Verification items for the finished model (mm, model axes). Give positions to 0.01 mm unless a question says otherwise; leave off trailing zeros. Write each loop counter-clockwise with the first axis right and the second up, starting at its lowest first coordinate (ties: lowest second). Pieces come first, ordered by that corner, then holes. Notation, with made-up numbers: (83, -19.5) - (88, -19.5) arc R30 ccw to (88, 3.5) - close; hole circle Ø2 at (29, -4.75). An arc over 180 degrees is marked (long way). Answer as a JSON object with one key per item and string values. Group by question number.
Item 1: Sectioned sample at A-A, the plane z = 85. Record the boundary of the cut face in (x, y), and give its area (3 significant figures).
Item 2: Go/stop test with flat-tipped pins: pin 1 (1.5 mm diameter, centred on y = 2.5, z = 78.5, fed in from +X); pin 2 (4.5 mm diameter, centred on y = 0, z = 25, fed in from -X); pin 3 (4 mm diameter, centred on x = -15.5, y = -1.5, fed in from +Z). Record where each tip stops, or that it passes through.
Item 3: Scan lines: line 1 along Y through (x, z) = (1, 25); line 2 along Z through (x, y) = (-11.5, -3.75); line 3 along X through (y, z) = (4.5, 12.5). Record each from-to range of solid material in increasing order. Write a range as [from, to].
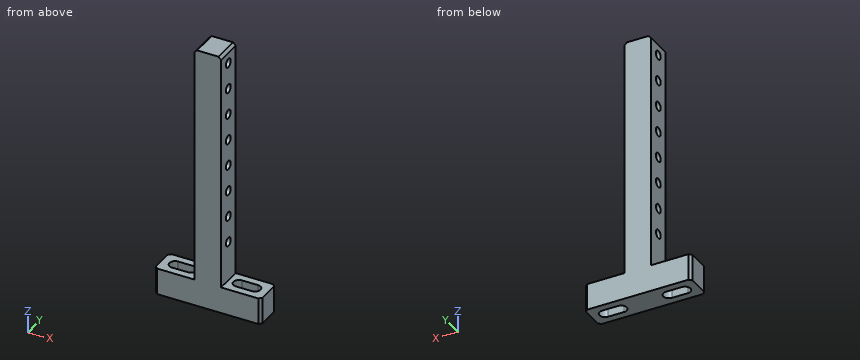
```python
from build123d import *

# Parameters (mm, degrees)
SKETCH1_W           = 40
SKETCH1_H           = 10
BOSS_EXTRUDE1_DEPTH = 10
SKETCH2_W           = 10
SKETCH2_H           = 10
BOSS_EXTRUDE2_DEPTH = 90
CUT_EXTRUDE1_DEPTH  = 103.102889283
M4_TAPPED_HOLE1_D   = 3.3
CHAMFER1_SIZE       = 1


with BuildPart() as part:
    # Sketch1 → Boss-Extrude1 (new body)
    with BuildSketch(Plane.XY):
        Rectangle(SKETCH1_W, SKETCH1_H)
    extrude(amount=BOSS_EXTRUDE1_DEPTH)

    # Sketch2 → Boss-Extrude2 (add)
    with BuildSketch(Plane.XY.offset(10)):
        Rectangle(SKETCH2_W, SKETCH2_H)
    extrude(amount=BOSS_EXTRUDE2_DEPTH)

    # Sketch3 → Cut-Extrude1 (cut, through all)
    with BuildSketch(Plane(origin=(0, 0, 0), x_dir=(-1, 0, 0), z_dir=(0, 0, -1))):
        with BuildLine():
            Line((-15, 2.1), (-9, 2.1))
            ThreePointArc((-9, 2.1), (-6.9, 0), (-9, -2.1))
            Line((-9, -2.1), (-15, -2.1))
            ThreePointArc((-15, -2.1), (-17.1, 0), (-15, 2.1))
        make_face()
        with BuildLine():
            Line((15, 2.1), (9, 2.1))
            ThreePointArc((9, 2.1), (6.9, 0), (9, -2.1))
            Line((9, -2.1), (15, -2.1))
            ThreePointArc((15, -2.1), (17.1, 0), (15, 2.1))
        make_face()
    extrude(amount=-CUT_EXTRUDE1_DEPTH, mode=Mode.SUBTRACT)

    # M4 Tapped Hole1 (through all)
    with Locations(Plane(origin=(5, 0, 0), x_dir=(0, 0, -1), z_dir=(1, 0, 0))):
        with Locations((-25, 0), (-35, 0), (-45, 0), (-55, 0), (-65, 0), (-75, 0), (-85, 0), (-95, 0)):
            Hole(M4_TAPPED_HOLE1_D / 2)

    # Chamfer1
    chamfer1_edges = [part.edges().sort_by_distance(p)[0] for p in [
        (20, 5, 5),
        (20, -5, 5),
        (-20, -5, 5),
        (-20, 5, 5),
        (5, 0, 100),
        (-5, 0, 100),
    ]]
    chamfer(chamfer1_edges, length=CHAMFER1_SIZE)


solid = part.part
```
Geometry check:
{
 "1": {"outline": "(-5, -5) - (5, -5) - (5, -1.65) - (-5, -1.65) - close; (-5, 1.65) - (5, 1.65) - (5, 5) - (-5, 5) - close", "area": "67.0 mm^2"},
 "2": {"pin 1": "x = 5", "pin 2": "x = -5", "pin 3": "z = 10"},
 "3": {"line 1": "[-5, -1.65], [1.65, 5]", "line 2": "[0, 10]", "line 3": "[-5, 5]"}
}
